The drawing under review shows one solid part. Ordinate dimensions are in mm from its lowest x, y, z. A direction names the side the tool comes from. Give positions to 0.01 mm unless a question says otherwise; leave off trailing zeros. Loops run counter-clockwise (first coordinate to the right, second up) from the corner with the lowest first, then second, coordinate; pieces in that order, holes last. Notation, with made-up numbers: (15, 87.25) -> (46, 87.25) arc R15 ccw to (46, 115.25) -> close; hole circle Ø11 at (-21.5, 84). An arc over 180 degrees is marked (long way). Answer in a Markdown table with one row per item. Add a question column.
(1) Consider section A-A on x = 16. Write out the cut boundary in (y, z), then the cut area to 3 significant figures.
(2) Consider section D-D on y = 16.75. Write out the cut boundary in (x, z).
(3) For the marked faces 1 and 2, list the 3-axis set-ups (+Z, -Z, +X, -X, +Y, -Y) from which the entire face can be reached by the end or side of a thin tool; tool diameter is ignored.
(4) For line 1 (Y direction, x = 10, z = 4); line 2 (X direction, y = 11.75, z = 1.9); line 3 (Z direction, x = 1.25, y = 7.5), list the stretches that pass through material, from the lowest coordinate up.
(5) Draft analysis for pull direction Y (two halves, no side actions). For the marked faces 3, 4 and 5, state which applies: +Y half, -Y half, draft (parallel to the pull), parting line (faces both ways), or undercut.
(6) Consider section C-C on z = 0.65. Write out the cut boundary in (x, y).
(7) For pin 1 (1.5 mm diameter, centred on x = 9, z = 1, fed in from -Y), flat-tipped, find the tip position at first contact; note if it passes through.
(8) Consider section B-B on x = 8.75. Write out the cut boundary in (y, z).
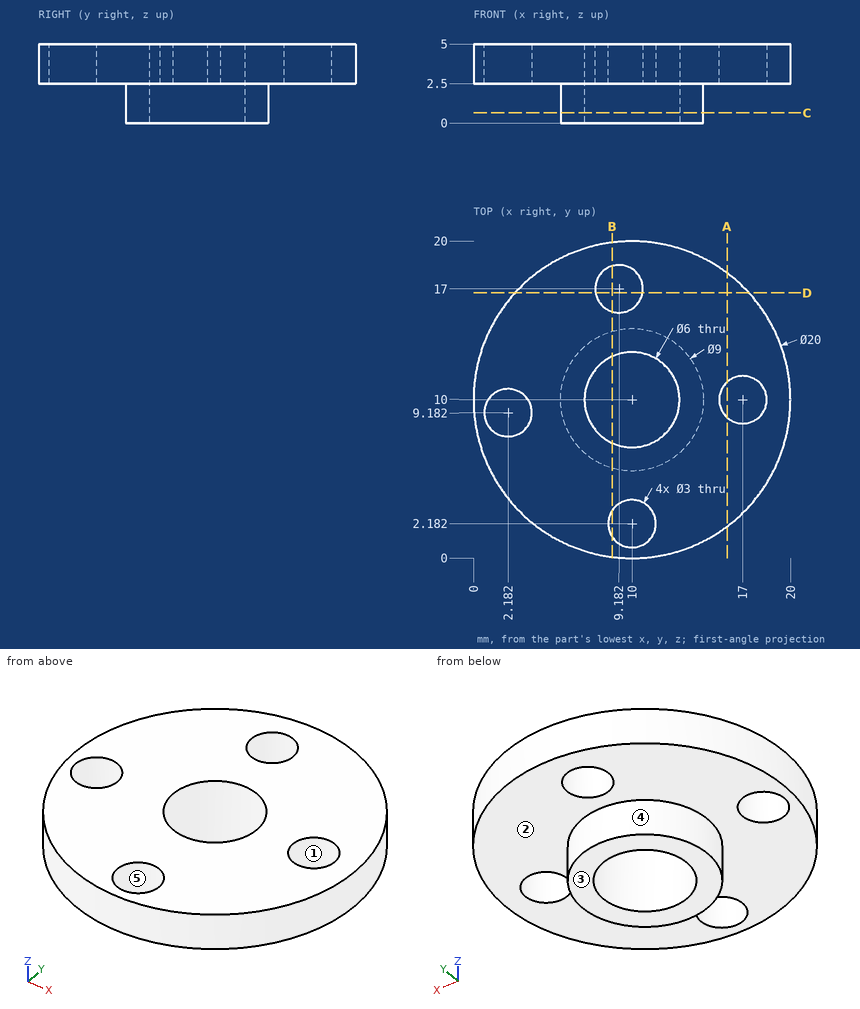
Values follow:
| question | item | result |
|---|---|---|
| 1 | outline | (2, 2.5) -> (8.88, 2.5) -> (8.88, 5) -> (2, 5) -> close; (11.12, 2.5) -> (18, 2.5) -> (18, 5) -> (11.12, 5) -> close |
| 1 | area | 34.4 mm2 |
| 2 | outline | (2.62, 2.5) -> (7.7, 2.5) -> (7.7, 5) -> (2.62, 5) -> close; (10.66, 2.5) -> (17.38, 2.5) -> (17.38, 5) -> (10.66, 5) -> close |
| 3 | face 1 | +Z, -Z |
| 3 | face 2 | -Z |
| 4 | line 1 | 0 to 0.68, 3.68 to 7, 13 to 15.74, 18.26 to 20 |
| 4 | line 2 | 5.85 to 7.56, 12.44 to 14.15 |
| 4 | line 3 | 2.5 to 5 |
| 5 | face 3 | draft |
| 5 | face 4 | parting line |
| 5 | face 5 | undercut |
| 6 | outline | circle Ø9 at (10, 10); hole circle Ø6 at (10, 10) |
| 7 | pin 1 | y = 5.51 |
| 8 | outline | (0.08, 2.5) -> (1.35, 2.5) -> (1.35, 5) -> (0.08, 5) -> close; (3.01, 2.5) -> (5.68, 2.5) -> (5.68, 0) -> (7.27, 0) -> (7.27, 5) -> (3.01, 5) -> close; (12.73, 0) -> (14.32, 0) -> (14.32, 2.5) -> (15.56, 2.5) -> (15.56, 5) -> (12.73, 5) -> close; (18.44, 2.5) -> (19.92, 2.5) -> (19.92, 5) -> (18.44, 5) -> close |
